```python
from build123d import *

# Parameters (mm, degrees)
SKETCH_1_W          = 250
SKETCH_1_H          = 150
EXTRUDE_1_DEPTH     = 12
SKETCH_2_R          = 10
CUT_EXTRUDE_1_DEPTH = 2
CUT_EXTRUDE_2_REACH = 148.267
SKETCH_3_R          = 16


with BuildPart() as part:
    # 草图1 → 凸台-拉伸1 (new body)
    with BuildSketch(Plane(origin=(0, 0, 0), x_dir=(1, 0, 0), z_dir=(0, 1, 0))):
        Rectangle(SKETCH_1_W, SKETCH_1_H)
    extrude(amount=EXTRUDE_1_DEPTH)

    # 草图2 → 切除-拉伸1 (cut)
    with BuildSketch(Plane(origin=(0, 0, 0), x_dir=(-1, 0, 0), z_dir=(0, -1, 0))):
        with Locations(Location((-108, 58, 0), (0, 0, 90))):
            Circle(SKETCH_2_R)
        with Locations(Location((108, 58, 0), (0, 0, 90))):
            Circle(SKETCH_2_R)
        with Locations(Location((-108, -58, 0), (0, 0, 90))):
            Circle(SKETCH_2_R)
        with Locations(Location((108, -58, 0), (0, 0, 90))):
            Circle(SKETCH_2_R)
    extrude(amount=-CUT_EXTRUDE_1_DEPTH, mode=Mode.SUBTRACT)

    # 草图3 → 切除-拉伸2 (cut, up to next)
    with BuildSketch(Plane(origin=(0, 12, 0), x_dir=(1, 0, 0), z_dir=(0, 1, 0)), mode=Mode.PRIVATE) as cut_extrude_2_sk1:
        with Locations(Location((-65, 0, 0), (0, 0, 270))):
            Circle(SKETCH_3_R)
    cut_extrude_2_tool1 = extrude(cut_extrude_2_sk1.sketch, amount=-CUT_EXTRUDE_2_REACH, mode=Mode.PRIVATE) & part.part
    # 草图3 → 切除-拉伸2 (cut, up to next)
    with BuildSketch(Plane(origin=(0, 12, 0), x_dir=(1, 0, 0), z_dir=(0, 1, 0)), mode=Mode.PRIVATE) as cut_extrude_2_sk2:
        with Locations(Location((65, 0, 0), (0, 0, 270))):
            Circle(SKETCH_3_R)
    cut_extrude_2_tool2 = extrude(cut_extrude_2_sk2.sketch, amount=-CUT_EXTRUDE_2_REACH, mode=Mode.PRIVATE) & part.part
    add(cut_extrude_2_tool1.solids().sort_by_distance((-65, 12, 0))[0], mode=Mode.SUBTRACT)
    add(cut_extrude_2_tool2.solids().sort_by_distance((65, 12, 0))[0], mode=Mode.SUBTRACT)


solid = part.part
```
Verification items for the finished model (mm, model axes). A direction names the side the tool comes from. Coordinates: 2 decimals unless noted, no trailing zeros. Loops run counter-clockwise (first coordinate to the right, second up) from the corner with the lowest first, then second, coordinate; pieces in that order, holes last. Notation, with made-up numbers: (66, 28) -> (117, 28) arc R32 cw to (117, 61) -> close; hole circle Ø2 at (13, 81.5). An arc over 180 degrees is marked (long way). Answer in a Markdown table with one row per item. Add a question column.
1. Section check D-D, the plane x = 108. Enter the section's corners in (y, z), then the cut area to 3 significant figures.
2. Depth check by flat-ended pin: P1, Ø19, axis at x = -65, z = 0, coming from the -Y side; P2, Ø10, axis at x = -109, z = -54, coming from the -Y side. Enter the tip coordinate at first touch or a pass-through.
3. Section check B-B, the plane z = 0. Enter the section's corners in (x, y), then the cut area to 3 significant figures.
4. Draft check along X on faces 1 (the face through (125, 6, 1)), 2 (the face through (-101.24, 0.99, 65.37)), 3 (the face through (-2, 6, -75)). Enter one of: +X half, -X half, draft (parallel to the pull), parting line (faces both ways), or undercut.
5. Material ranges on probe 1 along X at (y, z) = (9.75, 0); probe 2 along X at (y, z) = (0.85, 58); probe 3 along Y at (x, z) = (-105, -63.5), recorded low to high. Write a range as [from, to].
6. Section check C-C, the plane y = 9.75. Enter the section's corners in (x, z), then the cut area to 3 significant figures.
7. Section check A-A, the plane x = -65. Enter the section's corners in (y, z).
8. Access from +Z, -Z, +X, -X, +Y, -Y to the whole of each face (thin tool, end or side, straight path). Record for faces 4 (the face through (-49.136, 6.084, -2.083)), 5 (the face through (-108, 2, -58)).
Derived:
| question | item | result |
|---|---|---|
| 1 | outline | (0, -75) -> (12, -75) -> (12, 75) -> (0, 75) -> (0, 68) -> (2, 68) -> (2, 48) -> (0, 48) -> (0, -48) -> (2, -48) -> (2, -68) -> (0, -68) -> close |
| 1 | area | 1,720 mm² |
| 2 | P1 | passes through |
| 2 | P2 | stops at y = 2 |
| 3 | outline | (-125, 0) -> (-81, 0) -> (-81, 12) -> (-125, 12) -> close; (-49, 0) -> (49, 0) -> (49, 12) -> (-49, 12) -> close; (81, 0) -> (125, 0) -> (125, 12) -> (81, 12) -> close |
| 3 | area | 2,230 mm² |
| 4 | face 1 | +X half |
| 4 | face 2 | undercut |
| 4 | face 3 | draft |
| 5 | probe 1 | x = [-125, -81], [-49, 49], [81, 125] |
| 5 | probe 2 | x = [-125, -118], [-98, 98], [118, 125] |
| 5 | probe 3 | y = [2, 12] |
| 6 | outline | (-125, -75) -> (125, -75) -> (125, 75) -> (-125, 75) -> close; hole circle Ø32 at (-65, 0); hole circle Ø32 at (65, 0) |
| 6 | area | 35,900 mm² |
| 7 | outline | (0, -75) -> (12, -75) -> (12, -16) -> (0, -16) -> close; (0, 16) -> (12, 16) -> (12, 75) -> (0, 75) -> close |
| 8 | face 4 | +Y, -Y |
| 8 | face 5 | -Y |
